```python
from build123d import *

# Parameters (mm, degrees)
SKETCH_1_W          = 126
SKETCH_1_H          = 25
EXTRUDE_1_DEPTH     = 6
CUT_EXTRUDE_1_DEPTH = 66.339498008
SKETCH_3_W          = 160
SKETCH_3_H          = 12.2
CUT_EXTRUDE_2_DEPTH = 2
CHAMFER_1_SIZE      = 2
HOLE_WIZARD_M5_1_D  = 4.2
SKETCH_8_W          = 42.808580858
SKETCH_8_H          = 66.158715872
SKETCH_8_W_2        = 29.187668767
SKETCH_8_H_2        = 70.606360636
CUT_EXTRUDE_5_DEPTH = 2


with BuildPart() as part:
    # 草图1 → 凸台-拉伸1 (new, symmetric)
    with BuildSketch(Plane(origin=(0, 0, 0), x_dir=(1, 0, 0), z_dir=(0, 1, 0))):
        Rectangle(SKETCH_1_W, SKETCH_1_H)
    extrude(amount=EXTRUDE_1_DEPTH, both=True)

    # 草图2 → 切除-拉伸1 (cut, through all)
    with BuildSketch(Plane(origin=(0, 6, 0), x_dir=(1, 0, 0), z_dir=(0, 1, 0))):
        with BuildLine():
            Line((-54.4, 5), (-54.4, -5))
            ThreePointArc((-54.4, -5), (-57, -7.6), (-59.6, -5))
            Line((-59.6, -5), (-59.6, 5))
            ThreePointArc((-59.6, 5), (-57, 7.6), (-54.4, 5))
        make_face()
    cut_extrude_1 = extrude(amount=-CUT_EXTRUDE_1_DEPTH, mode=Mode.SUBTRACT)

    # 镜向1: 切除-拉伸1 across plane
    add(cut_extrude_1.mirror(Plane(origin=(0, 0, 0), x_dir=(0, 0, 1), z_dir=(1, 0, 0))), mode=Mode.SUBTRACT)

    # 草图3 → 切除-拉伸2 (cut)
    with BuildSketch(Plane(origin=(0, 6, 0), x_dir=(1, 0, 0), z_dir=(0, 1, 0))):
        Rectangle(SKETCH_3_W, SKETCH_3_H)
    extrude(amount=-CUT_EXTRUDE_2_DEPTH, mode=Mode.SUBTRACT)

    # 倒角1
    chamfer_1_edges = [part.edges().sort_by_distance(p)[0] for p in [
        (63, 0, 12.5),
        (-63, 0, 12.5),
        (-63, 0, -12.5),
        (63, 0, -12.5),
    ]]
    chamfer(chamfer_1_edges, length=CHAMFER_1_SIZE)

    # M5 螺纹孔1 (through all)
    with Locations(Plane(origin=(0, 4, 0), x_dir=(1, 0, 0), z_dir=(0, 1, 0))):
        with Locations((-40, 0), (40, 0)):
            Hole(HOLE_WIZARD_M5_1_D / 2)

    # 草图8 → 切除-拉伸5 (cut)
    with BuildSketch(Plane(origin=(0, 6, 0), x_dir=(1, 0, 0), z_dir=(0, 1, 0))):
        with Locations((-72.404290429, 14.176867687)):
            Rectangle(SKETCH_8_W, SKETCH_8_H)
        with Locations((65.593834383, 18.207545755)):
            Rectangle(SKETCH_8_W_2, SKETCH_8_H_2)
    extrude(amount=-CUT_EXTRUDE_5_DEPTH, mode=Mode.SUBTRACT)


solid = part.part
```
Source: CAD feature listing. Evaluate the final solid. Frame: model axes, mm. A direction names the side the tool comes from. Give positions to 0.01 mm unless a question says otherwise; leave off trailing zeros. Write each loop counter-clockwise with the first axis right and the second up, starting at its lowest first coordinate (ties: lowest second). Pieces come first, ordered by that corner, then holes.
1. Section query D-D (x = -57). Return the cut outline in (y, z), then the cut area to 3 significant figures.
2. First-contact query: pin 1 (0.6 mm diameter, centred on y = 5, z = -8, fed in from +X); pin 2 (6.5 mm diameter, centred on x = -40, z = 0, fed in from +Y); pin 3 (1.6 mm diameter, centred on y = 5.5, z = 8, fed in from -X). Flat tips, straight axial feed; report the tip coordinate or a pass-through.
3. Access query for faces 4 (the face through (-51, 5, 9)), 5 (the face through (-63, -1, 0)), 6 (the face through (59.6, -1, 0)), 7 (the face through (62, -0.9, -11.5)), 8 (the face through (-1, 5, -6.1)). Directions: +Z, -Z, +X, -X, +Y, -Y. A direction counts if a zero-diameter tool reaches every point of the face in a straight line with its end or side. Return the directions, or none.
4. Section query B-B (y = 2). Return the cut outline in (x, z).
5. Section query C-C (z = 0). Return the cut outline in (x, y), then the cut area to 3 significant figures.
6. Material intervals for line 1 along X through (y, z) = (2, -0.25); line 2 along X through (y, z) = (1, -3.5); line 3 along Z through (x, y) = (-40, -0.75), sorted ascending.
7. Section query A-A (x = 40). Return the cut outline in (y, z).
8. Pull-direction query (Z, two-part tool) for faces 1 (the face through (-1, 4, 0)), 2 (the face through (-1, -6, 0)), 3 (the face through (-1, 0, -12.5)); classes: +Z half, -Z half, draft (parallel to the pull), parting line (faces both ways), or undercut.
Output values:
1. outline: (-6, -12.5) - (4, -12.5) - (4, -7.6) - (-6, -7.6) - close; (-6, 7.6) - (4, 7.6) - (4, 12.5) - (-6, 12.5) - close
1. area: 98.0 mm2
2. pin 1: stops at x = 51
2. pin 2: stops at y = 4
2. pin 3: stops at x = -51
3. face 4: +Z, -Z, -X, +Y
3. face 5: +Z, -Z, -X, +Y, -Y
3. face 6: +Y, -Y
3. face 7: -Z, +X, +Y, -Y
3. face 8: +X, -X, +Y
4. outline: (-63, -10.5) - (-61, -12.5) - (61, -12.5) - (63, -10.5) - (63, 10.5) - (61, 12.5) - (-61, 12.5) - (-63, 10.5) - close; hole (-59.6, -5) arc R2.6 ccw to (-54.4, -5) - (-54.4, 5) arc R2.6 ccw to (-59.6, 5) - close; hole circle Ø4.2 at (-40, 0); hole circle Ø4.2 at (40, 0); hole (54.4, -5) arc R2.6 ccw to (59.6, -5) - (59.6, 5) arc R2.6 ccw to (54.4, 5) - close
5. outline: (-63, -6) - (-59.6, -6) - (-59.6, 4) - (-63, 4) - close; (-54.4, -6) - (-42.1, -6) - (-42.1, 4) - (-54.4, 4) - close; (-37.9, -6) - (37.9, -6) - (37.9, 4) - (-37.9, 4) - close; (42.1, -6) - (54.4, -6) - (54.4, 4) - (42.1, 4) - close; (59.6, -6) - (63, -6) - (63, 4) - (59.6, 4) - close
5. area: 1,070 mm2
6. line 1: x = -63 to -59.6, -54.4 to -42.09, -37.91 to 37.91, 42.09 to 54.4, 59.6 to 63
6. line 2: x = -63 to -59.6, -54.4 to 54.4, 59.6 to 63
6. line 3: z = -12.5 to -2.1, 2.1 to 12.5
7. outline: (-6, -12.5) - (6, -12.5) - (6, -6.1) - (4, -6.1) - (4, -2.1) - (-6, -2.1) - close; (-6, 2.1) - (4, 2.1) - (4, 6.1) - (6, 6.1) - (6, 12.5) - (-6, 12.5) - close
8. face 1: undercut
8. face 2: draft
8. face 3: -Z half
